```python
from build123d import *

# Parameters (mm, degrees)
LINK_PROFILE_SKETCH_R        = 1.5
LINK_BAR_100_CTRS_2X_3_DEPTH = 5


with BuildPart() as part:
    # Link Profile Sketch → Link Bar 100 Ctrs 2xØ3 (new body)
    with BuildSketch(Plane.XY):
        with BuildLine():
            Line((-50, 3), (50, 3))
            ThreePointArc((50, 3), (53, 0), (50, -3))
            Line((50, -3), (-50, -3))
            ThreePointArc((-50, -3), (-53, 0), (-50, 3))
        make_face()
        with Locations((-50, 0)):
            Circle(LINK_PROFILE_SKETCH_R, mode=Mode.SUBTRACT)
        with Locations((50, 0)):
            Circle(LINK_PROFILE_SKETCH_R, mode=Mode.SUBTRACT)
    extrude(amount=LINK_BAR_100_CTRS_2X_3_DEPTH)


solid = part.part
```
Input: part model. Units: mm. Frame: model coordinates. Give positions to 0.01 mm unless a question says otherwise; leave off trailing zeros. Order: outer loops, then holes, each group sorted by start corner. A loop starts at its lowest first (then second) coordinate and runs counter-clockwise, first axis right, second up.
1. Section B-B on z = 4. Return the cut outline in (x, y).
Derived:
outline: (-50, -3) - (50, -3) arc R3 ccw to (50, 3) - (-50, 3) arc R3 ccw to start; hole circle Ø3 at (-50, 0); hole circle Ø3 at (50, 0)
2. Mould query, pull axis X, two halves, no side actions, for faces 1 (the cylindrical face through (-53, 0, 2)), 2 (the cylindrical face through (53, 0, 2)), 3 (the cylindrical face through (-51.5, 0.07, 2.46)), 4 (the flat face through (-1, 3, 2)). Classes: released by +X, released by -X, zero draft, split by the parting line, or undercut.
Derived:
face 1: released by -X
face 2: released by +X
face 3: undercut
face 4: zero draft
3. Material intervals for L1, parallel to X at y = 0.1, z = 2.95; L2, parallel to Y at x = -50, z = 2.25; L3, parallel to X at y = -0.95, z = 1.05, sorted ascending.
Derived:
L1: x = -53 to -51.5, -48.5 to 48.5, 51.5 to 53
L2: y = -3 to -1.5, 1.5 to 3
L3: x = -52.85 to -51.16, -48.84 to 48.84, 51.16 to 52.85
4. Section A-A on y = 0. Return the cut outline in (x, z), and give its area (3 significant figures).
Derived:
outline: (-53, 0) - (-51.5, 0) - (-51.5, 5) - (-53, 5) - close; (-48.5, 0) - (48.5, 0) - (48.5, 5) - (-48.5, 5) - close; (51.5, 0) - (53, 0) - (53, 5) - (51.5, 5) - close
area: 500 mm2
